Source: CAD feature listing. Evaluate the final solid. Frame: model axes, mm. Face numbers are marked on the shaded views. A direction names the side the tool comes from. Round coordinates to 2 decimals unless told otherwise and drop trailing zeros. Write each loop counter-clockwise with the first axis right and the second up, starting at its lowest first coordinate (ties: lowest second). Pieces come first, ordered by that corner, then holes. Notation, with made-up numbers: M 52,-39 L 83,-39 A6 ccw 83,-34 Z; hole C -31,62.5 d5. An arc over 180 degrees is marked long. Put each result on its own line as item: value. Start each with the question number.
```python
from build123d import *

# Parameters (mm, degrees)
MAIN_BODY_50MM_DEPTH     = 50
BEARING_SEAT_CUT_1_DEPTH = 10
BEARING_START            = -10
BEARING_SEAT_CUT_2_DEPTH = 10
TOP_GROOVE_CUT_1_DEPTH   = 10
TOP_START                = -10
TOP_GROOVE_CUT_2_DEPTH   = 10
BASE_NOTCH_1_SKETCH_W    = 7
BASE_NOTCH_1_SKETCH_H    = 30
BASE_NOTCH_CUT_1_DEPTH   = 10
BASE_NOTCH_2_SKETCH_W    = 7
BASE_NOTCH_2_SKETCH_H    = 30
BASE_NOTCH_CUT_2_DEPTH   = 10


with BuildPart() as part:
    # Body Profile Sketch → Main Body 50mm (new body)
    with BuildSketch(Plane.XY):
        Polygon((0, 0), (0, 5), (-25, 5), (-25, 15), (-10, 15), (-10, 65), (5, 65), (15, 75), (22.5, 75), (30, 75), (37.5, 75), (45, 75), (55, 65), (70, 65), (70, 15), (85, 15), (85, 5), (60, 5), (60, 0), (50, 0), (50, 20), (10, 20), (10, 0), align=None)
    extrude(amount=MAIN_BODY_50MM_DEPTH)

    # Bearing Seat 1 Sketch → Bearing Seat Cut 1 (cut)
    with BuildSketch(Plane.ZY.offset(10)):
        with BuildLine():
            Line((8, 65), (42, 65))
            ThreePointArc((42, 65), (25, 48), (8, 65))
        make_face()
    extrude(amount=-BEARING_SEAT_CUT_1_DEPTH, mode=Mode.SUBTRACT)

    # Bearing Seat 2 Sketch → Bearing Seat Cut 2 (cut)
    with BuildSketch(Plane(origin=(70, 0, 0), x_dir=(0, 0, -1), z_dir=(1, 0, 0)).offset(BEARING_START)):
        with BuildLine():
            Line((-42, 65), (-8, 65))
            ThreePointArc((-8, 65), (-25, 48), (-42, 65))
        make_face()
    extrude(amount=BEARING_SEAT_CUT_2_DEPTH, mode=Mode.SUBTRACT)

    # Top Groove 1 Sketch → Top Groove Cut 1 (cut)
    with BuildSketch(Plane(origin=(0, 0, 0), x_dir=(-1, 0, 0), z_dir=(0, 0, -1))):
        with BuildLine():
            Line((-30, 75), (-37.5, 75))
            Line((-37.5, 75), (-37.5, 55.618380291))
            ThreePointArc((-37.5, 55.618380291), (-30, 32), (-22.5, 55.618380291))
            Line((-22.5, 55.618380291), (-22.5, 75))
            Line((-22.5, 75), (-30, 75))
        make_face()
    extrude(amount=-TOP_GROOVE_CUT_1_DEPTH, mode=Mode.SUBTRACT)

    # Top Groove 2 Sketch → Top Groove Cut 2 (cut)
    with BuildSketch(Plane.XY.offset(50).offset(TOP_START)):
        with BuildLine():
            Line((30, 75), (22.5, 75))
            Line((22.5, 75), (22.5, 55.618380291))
            ThreePointArc((22.5, 55.618380291), (30, 32), (37.5, 55.618380291))
            Line((37.5, 55.618380291), (37.5, 75))
            Line((37.5, 75), (30, 75))
        make_face()
    extrude(amount=TOP_GROOVE_CUT_2_DEPTH, mode=Mode.SUBTRACT)

    # Base Notch 1 Sketch → Base Notch Cut 1 (cut)
    with BuildSketch(Plane(origin=(0, 15, 0), x_dir=(1, 0, 0), z_dir=(0, 1, 0))):
        with Locations((-21.5, -25)):
            Rectangle(BASE_NOTCH_1_SKETCH_W, BASE_NOTCH_1_SKETCH_H)
    extrude(amount=-BASE_NOTCH_CUT_1_DEPTH, mode=Mode.SUBTRACT)

    # Base Notch 2 Sketch → Base Notch Cut 2 (cut)
    with BuildSketch(Plane(origin=(0, 15, 0), x_dir=(1, 0, 0), z_dir=(0, 1, 0))):
        with Locations((81.5, -25)):
            Rectangle(BASE_NOTCH_2_SKETCH_W, BASE_NOTCH_2_SKETCH_H)
    extrude(amount=-BASE_NOTCH_CUT_2_DEPTH, mode=Mode.SUBTRACT)


solid = part.part
```
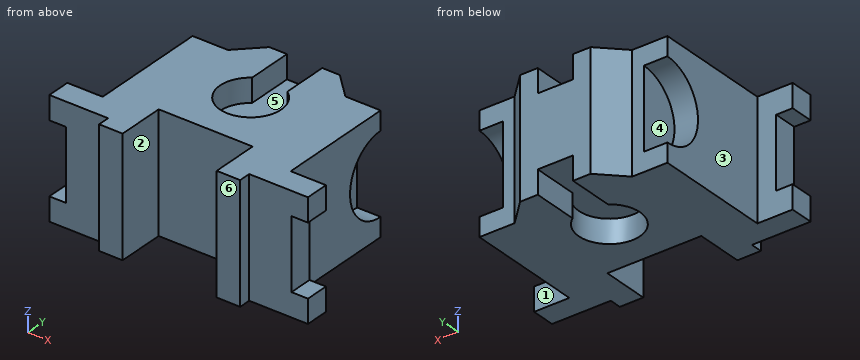
(1) Access query for the marked faces 1, 2 and 3. Directions: +Z, -Z, +X, -X, +Y, -Y. A direction counts if a zero-diameter tool reaches every point of the face in a straight line with its end or side. Return the directions, or none.
(2) Contact query for flat-ended pins moving along their axis: P1, Ø6, axis at x = -10.5, z = 8, coming from the -Y side; P2, Ø5, axis at y = 70, z = 43.5, coming from the -X side; P3, Ø11, axis at y = 8.5, z = 30, coming from the +X side. Output: stop coordinate, or through.
(3) Section query C-C (x = 30). Return loops of the section in (y, z), and give its area (3 significant figures).
(4) Section query A-A (y = 45). Return loops of the section in (x, z).
(5) Section query B-B (z = 25). Return loops of the section in (x, y), and give its area (3 significant figures).
(6) Ray query, line 1 along X through (y, z) = (45.5, 44); line 2 along X through (y, z) = (9, 31); line 3 along Y through (x, z) = (30, 44). Return the intervals inside material, ascending.
(7) Pull-direction query (Z, two-part tool) for the marked faces 4, 5 and 6; classes: +Z half, -Z half, draft (parallel to the pull), parting line (faces both ways), or undercut.
(8) Section query D-D (z = 30). Return loops of the section in (x, y).
Entries:
1. face 1: +Z, -Z, +X, +Y
1. face 2: +Z, -Z, -Y
1. face 3: +Z, -Z, -X, +Y
2. P1: y = 5
2. P2: x = 7.5
2. P3: x = 78
3. outline: M 20,0 L 32,0 L 32,10 L 75,10 L 75,40 L 32,40 L 32,50 L 20,50 Z
3. area: 1,890 mm2
4. outline: M -10,0 L 17,0 L 17,10 L 43,10 L 43,0 L 70,0 L 70,50 L 43,50 L 43,40 L 17,40 L 17,50 L -10,50 Z
5. outline: M -18,5 L 0,5 L 0,0 L 10,0 L 10,20 L 50,20 L 50,0 L 60,0 L 60,5 L 78,5 L 78,15 L 70,15 L 70,48 L 60,48 L 60,65 L 55,65 L 45,75 L 15,75 L 5,65 L 0,65 L 0,48 L -10,48 L -10,15 L -18,15 Z
5. area: 4,520 mm2
6. line 1: -10 to 17.01, 42.99 to 70
6. line 2: -18 to 10, 50 to 78
6. line 3: 20 to 32
7. face 4: undercut
7. face 5: +Z half
7. face 6: draft
8. outline: M -18,5 L 0,5 L 0,0 L 10,0 L 10,20 L 50,20 L 50,0 L 60,0 L 60,5 L 78,5 L 78,15 L 70,15 L 70,48.75 L 60,48.75 L 60,65 L 55,65 L 45,75 L 15,75 L 5,65 L 0,65 L 0,48.75 L -10,48.75 L -10,15 L -18,15 Z
